Verification items for the finished model (mm, model axes). A direction names the side the tool comes from. Round coordinates to 2 decimals unless told otherwise and drop trailing zeros. Write each loop counter-clockwise with the first axis right and the second up, starting at its lowest first coordinate (ties: lowest second). Pieces come first, ordered by that corner, then holes. Notation, with made-up numbers: (27.5, 35.25) - (40.5, 35.25) arc R16 cw to (40.5, 58.25) - close; hole circle Ø6 at (75.25, -19.5). An arc over 180 degrees is marked (long way). Write each question's results on one line, items separated by ' | '.
```python
from build123d import *

# Parameters (mm, degrees)
SKETCH1_W                      = 400
SKETCH1_H                      = 100
BOSS_EXTRUDE1_DEPTH            = 12
SKETCH2_W                      = 100
SKETCH2_H                      = 12
BOSS_EXTRUDE2_DEPTH            = 40
CUT_EXTRUDE1_DEPTH             = 4
M8_TAPPED_HOLE2_D              = 6.8
M8_TAPPED_HOLE2_DEPTH          = 22
M8_TAPPED_HOLE2_TIP            = 2.042926105
M5_TAPPED_HOLE1_D              = 4.2
M5_TAPPED_HOLE1_DEPTH          = 12.4
M5_TAPPED_HOLE1_TIP            = 1.2618073
M4_TAPPED_HOLE1_D              = 3.3
M4_TAPPED_HOLE1_DEPTH          = 10.1
M4_TAPPED_HOLE1_TIP            = 0.991420021
SKETCH10_R                     = 2
CUT_EXTRUDE2_DEPTH             = 220.645168397
M8_TAPPED_HOLE1_D              = 6.8
M8_TAPPED_HOLE1_DEPTH          = 19.75
M8_TAPPED_HOLE1_TIP            = 2.042926105
F_5_5_5_5_DIAMETER_HOLE1_D     = 5.5
F_5_5_5_5_DIAMETER_HOLE1_DEPTH = 76
F_5_5_5_5_DIAMETER_HOLE1_TIP   = 1.652366702
CUT_EXTRUDE3_DEPTH             = 220.645168397
CHAMFER1_SIZE                  = 5
FILLET1_R                      = 10
CUT_EXTRUDE4_DEPTH             = 220.645168397


with BuildPart() as part:
    # Sketch1 → Boss-Extrude1 (new body)
    with BuildSketch(Plane.XY):
        Rectangle(SKETCH1_W, SKETCH1_H)
    extrude(amount=BOSS_EXTRUDE1_DEPTH)

    # Sketch2 → Boss-Extrude2 (add)
    with BuildSketch(Plane(origin=(0, 50, 0), x_dir=(1, 0, 0), z_dir=(0, 1, 0))):
        with Locations((150, -6)):
            Rectangle(SKETCH2_W, SKETCH2_H)
    extrude(amount=BOSS_EXTRUDE2_DEPTH)

    # Sketch3 → Cut-Extrude1 (cut)
    with BuildSketch(Plane.XY.offset(12)):
        with BuildLine():
            Line((4, 50), (4, -10))
            ThreePointArc((4, -10), (0, -14), (-4, -10))
            Line((-4, -10), (-4, 50))
            ThreePointArc((-4, 50), (0, 54), (4, 50))
        make_face()
    extrude(amount=-CUT_EXTRUDE1_DEPTH, mode=Mode.SUBTRACT)

    # M8 Tapped Hole2
    with Locations(Plane(origin=(0, -50, 0), x_dir=(-1, 0, 0), z_dir=(0, -1, 0))):
        with Locations((0, -6)):
            Hole(M8_TAPPED_HOLE2_D / 2, depth=M8_TAPPED_HOLE2_DEPTH)
            with Locations((0, 0, -(M8_TAPPED_HOLE2_DEPTH + M8_TAPPED_HOLE2_TIP / 2))):  # 118° drill point
                Cone(0, M8_TAPPED_HOLE2_D / 2, M8_TAPPED_HOLE2_TIP, mode=Mode.SUBTRACT)

    # M5 Tapped Hole1
    with Locations(Plane(origin=(0, 0, 0), x_dir=(-1, 0, 0), z_dir=(0, 0, -1))):
        with Locations((22.5, -16), (22.5, -44)):
            Hole(M5_TAPPED_HOLE1_D / 2, depth=M5_TAPPED_HOLE1_DEPTH)
            with Locations((0, 0, -(M5_TAPPED_HOLE1_DEPTH + M5_TAPPED_HOLE1_TIP / 2))):  # 118° drill point
                Cone(0, M5_TAPPED_HOLE1_D / 2, M5_TAPPED_HOLE1_TIP, mode=Mode.SUBTRACT)

    # M4 Tapped Hole1
    with Locations(Plane(origin=(0, 0, 0), x_dir=(-1, 0, 0), z_dir=(0, 0, -1))):
        with Locations((180, 25), (140, 25), (100, 25), (60, 25), (20, 25), (-20, 25)):
            Hole(M4_TAPPED_HOLE1_D / 2, depth=M4_TAPPED_HOLE1_DEPTH)
            with Locations((0, 0, -(M4_TAPPED_HOLE1_DEPTH + M4_TAPPED_HOLE1_TIP / 2))):  # 118° drill point
                Cone(0, M4_TAPPED_HOLE1_D / 2, M4_TAPPED_HOLE1_TIP, mode=Mode.SUBTRACT)

    # Sketch10 → Cut-Extrude2 (cut, through all)
    with BuildSketch(Plane(origin=(0, 0, 0), x_dir=(-1, 0, 0), z_dir=(0, 0, -1))):
        with Locations((180, 39)):
            Circle(SKETCH10_R)
        with Locations((-20, 39)):
            Circle(SKETCH10_R)
    extrude(amount=-CUT_EXTRUDE2_DEPTH, mode=Mode.SUBTRACT)

    # M8 Tapped Hole1
    with Locations(Plane(origin=(0, 0, 0), x_dir=(-1, 0, 0), z_dir=(0, 0, -1))):
        with Locations((50, -30), (50, 30), (-50, -30), (-50, 30)):
            Hole(M8_TAPPED_HOLE1_D / 2, depth=M8_TAPPED_HOLE1_DEPTH)
            with Locations((0, 0, -(M8_TAPPED_HOLE1_DEPTH + M8_TAPPED_HOLE1_TIP / 2))):  # 118° drill point
                Cone(0, M8_TAPPED_HOLE1_D / 2, M8_TAPPED_HOLE1_TIP, mode=Mode.SUBTRACT)

    # Ø5.5 (5.5) Diameter Hole1
    with Locations(Plane.XY.offset(12)):
        with Locations((120, 75), (180, 75), (150, 25)):
            Hole(F_5_5_5_5_DIAMETER_HOLE1_D / 2, depth=F_5_5_5_5_DIAMETER_HOLE1_DEPTH)
            with Locations((0, 0, -(F_5_5_5_5_DIAMETER_HOLE1_DEPTH + F_5_5_5_5_DIAMETER_HOLE1_TIP / 2))):  # 118° drill point
                Cone(0, F_5_5_5_5_DIAMETER_HOLE1_D / 2, F_5_5_5_5_DIAMETER_HOLE1_TIP, mode=Mode.SUBTRACT)

    # Sketch15 → Cut-Extrude3 (cut, through all)
    with BuildSketch(Plane.XY.offset(12)):
        with BuildLine():
            Line((122.75, 77.5), (122.75, 72.5))
            ThreePointArc((122.75, 72.5), (120, 69.75), (117.25, 72.5))
            Line((117.25, 72.5), (117.25, 77.5))
            ThreePointArc((117.25, 77.5), (120, 80.25), (122.75, 77.5))
        make_face()
        with BuildLine():
            Line((182.75, 77.5), (182.75, 72.5))
            ThreePointArc((182.75, 72.5), (180, 69.75), (177.25, 72.5))
            Line((177.25, 72.5), (177.25, 77.5))
            ThreePointArc((177.25, 77.5), (180, 80.25), (182.75, 77.5))
        make_face()
        with BuildLine():
            Line((155.25, 27.5), (155.25, 22.5))
            ThreePointArc((155.25, 22.5), (150, 17.25), (144.75, 22.5))
            Line((144.75, 22.5), (144.75, 27.5))
            ThreePointArc((144.75, 27.5), (150, 32.75), (155.25, 27.5))
        make_face()
    extrude(amount=-CUT_EXTRUDE3_DEPTH, mode=Mode.SUBTRACT)

    # Chamfer1
    chamfer1_edges = [part.edges().sort_by_distance(p)[0] for p in [
        (100, 90, 6),
        (200, 90, 6),
        (200, -50, 6),
        (-200, 50, 6),
        (-200, -50, 6),
    ]]
    chamfer(chamfer1_edges, length=CHAMFER1_SIZE)

    # Fillet1
    fillet1_edges = [part.edges().sort_by_distance(p)[0] for p in [
        (100, 50, 6),
    ]]
    fillet(fillet1_edges, radius=FILLET1_R)

    # Sketch16 → Cut-Extrude4 (cut, through all)
    with BuildSketch(Plane(origin=(0, 0, 0), x_dir=(-1, 0, 0), z_dir=(0, 0, -1))):
        with BuildLine():
            Line((-132, 72.5), (-132, 77.5))
            ThreePointArc((-132, 77.5), (-130, 79.5), (-128, 77.5))
            Line((-128, 77.5), (-128, 72.5))
            ThreePointArc((-128, 72.5), (-130, 70.5), (-132, 72.5))
        make_face()
        with BuildLine():
            Line((-172, 72.5), (-172, 77.5))
            ThreePointArc((-172, 77.5), (-170, 79.5), (-168, 77.5))
            Line((-168, 77.5), (-168, 72.5))
            ThreePointArc((-168, 72.5), (-170, 70.5), (-172, 72.5))
        make_face()
    extrude(amount=-CUT_EXTRUDE4_DEPTH, mode=Mode.SUBTRACT)


solid = part.part
```
(1) Set-up check for faces 1 (the cylindrical face through (149.88, 32.75, 6.08)), 2 (the flat face through (149, 90, 6)), 3 (the flat face through (-54, 50, 6)): record each of +Z, -Z, +X, -X, +Y, -Y from which the full face is reachable in a straight line by a thin tool's end or side.
Answer:
face 1: +Z, -Z | face 2: +Z, -Z, +X, -X, +Y | face 3: +Z, -Z, -X, +Y
(2) Thickness scan on L1, parallel to Y at x = -22.5, z = 4; L2, parallel to X at y = 72.5, z = 6.75; L3, parallel to X at y = -39, z = 6.5. Record the ranges inside material, lowest first.
Answer:
L1: -50 to -46.1, -41.9 to -18.1, -13.9 to 50 | L2: 100 to 117.25, 122.75 to 128, 132 to 168, 172 to 177.25, 182.75 to 200 | L3: -200 to -3.36, 3.36 to 200
(3) Mould release check, pull along Z, two halves, no side actions. Record for faces 4 (the cylindrical face through (-0.44, -38.85, 2.63)), 5 (the flat face through (-3, -50, 3)), 6 (the flat face through (0, 18, 8)), 7 (the flat face through (-3, 3, 0)): released by +Z, released by -Z, zero draft, split by the parting line, or undercut.
Answer:
face 4: undercut | face 5: zero draft | face 6: released by +Z | face 7: released by -Z
(4) Go/stop test with flat-tipped pins: pin 1 Ø8 at (x, y) = (-91, 28.5) entering from -Z; pin 2 Ø4 at (y, z) = (75.5, 8) entering from -X; pin 3 Ø4 at (x, z) = (0, 6) entering from +Y; pin 4 Ø6.5 at (x, y) = (0, 13.5) entering from +Z. Record where each tip stops, or that it passes through.
Answer:
pin 1: z = 0 | pin 2: x = 100 | pin 3: y = 50 | pin 4: z = 8
(5) Section check A-A (x = -94.5). Record the cut outline in (y, z), plus the area to 3 significant figures.
Answer:
outline: (-50, 0) - (50, 0) - (50, 12) - (-50, 12) - close | area: 1,200 mm2
